```python
from build123d import *


with BuildPart() as part:
    # Sketch1 → Revolve1 (revolve)
    with BuildSketch(Plane.XY, mode=Mode.PRIVATE) as revolve1_sk:
        with BuildLine():
            Line((-2.8, 0), (-3.463509174, 0))
            ThreePointArc((-3.463509174, 0), (-5.131546288, -0.236524296), (-6.668072967, -0.927449272))
            Line((-6.668072967, -0.927449272), (-10.031927033, -3.052550728))
            ThreePointArc((-10.031927033, -3.052550728), (-11.568453712, -3.743475704), (-13.236490826, -3.98))
            Line((-13.236490826, -3.98), (-13.9, -3.98))
            Line((-13.9, -3.98), (-13.9, -5.98))
            Line((-13.9, -5.98), (-13.236490826, -5.98))
            ThreePointArc((-13.236490826, -5.98), (-11.568453712, -5.743475704), (-10.031927033, -5.052550728))
            Line((-10.031927033, -5.052550728), (-6.668072967, -2.927449272))
            ThreePointArc((-6.668072967, -2.927449272), (-5.131546288, -2.236524296), (-3.463509174, -2))
            Line((-3.463509174, -2), (-2.8, -2))
            Line((-2.8, -2), (-2.8, 0))
        make_face()
    revolve(revolve1_sk.sketch.rotate(Axis((0, 0, 0), (0, -1, 0)), 270), axis=Axis((0, 0, 0), (0, -1, 0)))


solid = part.part
```
Build history of the part. All positions in model axes, mm. Give positions to 0.01 mm unless a question says otherwise; leave off trailing zeros. Loops run counter-clockwise (first coordinate to the right, second up) from the corner with the lowest first, then second, coordinate; pieces in that order, holes last.
Item 1: Flat gauge pins, fed straight in: pin 1 (3 mm diameter, centred on x = -7, y = -4.5, fed in from +Z); pin 2 (2 mm diameter, centred on y = -1.5, z = 0.5, fed in from +X); pin 3 (1.5 mm diameter, centred on x = -2.5, z = 10, fed in from -Y). Where does each tip first touch, or does it go through?
Answers follow:
pin 1: stops at z = 12.77
pin 2: stops at x = 9.14
pin 3: stops at y = -5.57
Item 2: Slice it at B-B, the plane y = -3.65. List the corners of the cut face in (x, z), and give its area (3 significant figures).
Answers follow:
outline: circle Ø22.55 at (0, 0); hole circle Ø15.62 at (0, 0)
area: 208 mm2
Item 3: Drill centre lines: line 1 (X direction, y = -0.7, z = 2.5); line 2 (X direction, y = -5, z = 4); line 3 (Y direction, x = 3, z = -1.5). Where is each one in solid material? Low to high.
Answers follow:
line 1: x = -5.76 to -1.26, 1.26 to 5.76
line 2: x = -13.31 to -9.11, 9.11 to 13.31
line 3: y = -2 to 0
Item 4: Slice it at A-A, the plane y = -5.5. List the corners of the cut face in (x, z).
Answers follow:
outline: circle Ø27.8 at (0, 0); hole circle Ø21.77 at (0, 0)
Item 5: Pull direction X, two halves, no side cores. Call faces 1 (the face through (0, 0, -3)), 2 (the face through (13.57, -4.99, -3.01)), 3 (the face through (0, -2, 3)): released by +X, released by -X, zero draft, split by the parting line, or undercut.
Answers follow:
face 1: zero draft
face 2: split by the parting line
face 3: undercut
